Build history of the part. All positions in model axes, mm. Round coordinates to 2 decimals unless told otherwise and drop trailing zeros. Write each loop counter-clockwise with the first axis right and the second up, starting at its lowest first coordinate (ties: lowest second). Pieces come first, ordered by that corner, then holes.
1) Wall check: probe 1 along Z at (x, y) = (6, -0.75); probe 2 along X at (y, z) = (1.35, 1.95); probe 3 along X at (y, z) = (0.85, 1.15). Give the ranges that are in metal, low to high.
2) Flat gauge pin, fed straight in: pin 1 (1 mm diameter, centred on x = 5, z = 0.5, fed in from +Y). Where does the tip first touch, or does it go through?
3) Saw through at A-A (z = 1.8). Write the cut outline in (x, y).
from build123d import *

# Parameters (mm, degrees)
BASE_EXTRUDE_DEPTH = 5
FILLET1_R          = 0.4


with BuildPart() as part:
    # Sketch1 → Base-Extrude (new body)
    with BuildSketch(Plane.XY):
        with BuildLine():
            Line((-4, 2.5), (4, 2.5))
            ThreePointArc((4, 2.5), (6.5, 0), (4, -2.5))
            Line((4, -2.5), (-4, -2.5))
            ThreePointArc((-4, -2.5), (-6.5, 0), (-4, 2.5))
        make_face()
    extrude(amount=BASE_EXTRUDE_DEPTH)

    # Fillet1
    fillet1_edges = [part.edges().sort_by_distance(p)[0] for p in [
        (6.5, 0, 5),
        (0, 2.5, 5),
        (-6.5, 0, 5),
        (0, 2.5, 0),
        (6.5, 0, 0),
        (0, -2.5, 0),
        (-6.5, 0, 0),
        (0, -2.5, 5),
    ]]
    fillet(fillet1_edges, radius=FILLET1_R)


solid = part.part
Evaluation:
1. probe 1: z = 0 to 5
1. probe 2: x = -6.1 to 6.1
1. probe 3: x = -6.35 to 6.35
2. pin 1: stops at y = 2.45
3. outline: (-4, -2.5) - (4, -2.5) arc R2.5 ccw to (4, 2.5) - (-4, 2.5) arc R2.5 ccw to start
